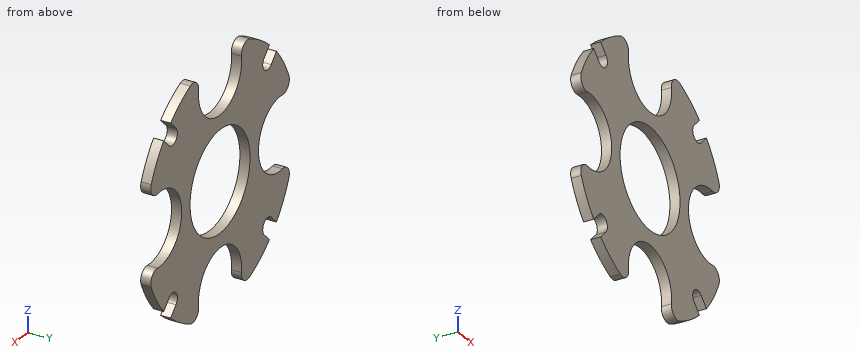
```python
from build123d import *

# Parameters (mm, degrees)
SKETCH4_R           = 5
BOSS_EXTRUDE1_DEPTH = 1


with BuildPart() as part:
    # Sketch4 → Boss-Extrude1 (new body)
    with BuildSketch(Plane(origin=(0, 0, 0), x_dir=(1, 0, 0), z_dir=(0, 1, 0))):
        with BuildLine():
            Line((-7.353910524, -8.520636713), (-8.236199678, -9.402925867))
            ThreePointArc((-8.236199678, -9.402925867), (-6.68048223, -10.565091442), (-4.963540243, -11.472282609))
            ThreePointArc((-4.963540243, -11.472282609), (-3.967940107, -11.355610167), (-3.573748975, -10.433956522))
            ThreePointArc((-3.573748975, -10.433956522), (0, -6.4), (3.573748975, -10.433956522))
            ThreePointArc((3.573748975, -10.433956522), (3.967940107, -11.355610167), (4.963540243, -11.472282609))
            ThreePointArc((4.963540243, -11.472282609), (6.68048223, -10.565091442), (8.236199678, -9.402925867))
            Line((8.236199678, -9.402925867), (7.353910524, -8.520636713))
            ThreePointArc((7.353910524, -8.520636713), (7.353910524, -7.353910524), (8.520636713, -7.353910524))
            Line((8.520636713, -7.353910524), (9.402925867, -8.236199678))
            ThreePointArc((9.402925867, -8.236199678), (10.565091442, -6.68048223), (11.472282609, -4.963540243))
            ThreePointArc((11.472282609, -4.963540243), (11.355610167, -3.967940107), (10.433956522, -3.573748975))
            ThreePointArc((10.433956522, -3.573748975), (6.4, 0), (10.433956522, 3.573748975))
            ThreePointArc((10.433956522, 3.573748975), (11.355610167, 3.967940107), (11.472282609, 4.963540243))
            ThreePointArc((11.472282609, 4.963540243), (10.565091442, 6.68048223), (9.402925867, 8.236199678))
            Line((9.402925867, 8.236199678), (8.520636713, 7.353910524))
            ThreePointArc((8.520636713, 7.353910524), (7.353910524, 7.353910524), (7.353910524, 8.520636713))
            Line((7.353910524, 8.520636713), (8.236199678, 9.402925867))
            ThreePointArc((8.236199678, 9.402925867), (6.68048223, 10.565091442), (4.963540243, 11.472282609))
            ThreePointArc((4.963540243, 11.472282609), (3.967940107, 11.355610167), (3.573748975, 10.433956522))
            ThreePointArc((3.573748975, 10.433956522), (0, 6.4), (-3.573748975, 10.433956522))
            ThreePointArc((-3.573748975, 10.433956522), (-3.967940107, 11.355610167), (-4.963540243, 11.472282609))
            ThreePointArc((-4.963540243, 11.472282609), (-6.68048223, 10.565091442), (-8.236199678, 9.402925867))
            Line((-8.236199678, 9.402925867), (-7.353910524, 8.520636713))
            ThreePointArc((-7.353910524, 8.520636713), (-7.353910524, 7.353910524), (-8.520636713, 7.353910524))
            Line((-8.520636713, 7.353910524), (-9.402925867, 8.236199678))
            ThreePointArc((-9.402925867, 8.236199678), (-10.565091442, 6.68048223), (-11.472282609, 4.963540243))
            ThreePointArc((-11.472282609, 4.963540243), (-11.355610167, 3.967940107), (-10.433956522, 3.573748975))
            ThreePointArc((-10.433956522, 3.573748975), (-6.4, 0), (-10.433956522, -3.573748975))
            ThreePointArc((-10.433956522, -3.573748975), (-11.355610167, -3.967940107), (-11.472282609, -4.963540243))
            ThreePointArc((-11.472282609, -4.963540243), (-10.565091442, -6.68048223), (-9.402925867, -8.236199678))
            Line((-9.402925867, -8.236199678), (-8.520636713, -7.353910524))
            ThreePointArc((-8.520636713, -7.353910524), (-7.353910524, -7.353910524), (-7.353910524, -8.520636713))
        make_face()
        with Locations(Location((0, 0, 0), (0, 0, 90))):
            Circle(SKETCH4_R, mode=Mode.SUBTRACT)
    extrude(amount=BOSS_EXTRUDE1_DEPTH)


solid = part.part
```
Source: CAD feature listing. Evaluate the final solid. Frame: model axes, mm. Coordinates: 2 decimals unless noted, no trailing zeros. Loops run counter-clockwise (first coordinate to the right, second up) from the corner with the lowest first, then second, coordinate; pieces in that order, holes last. Notation, with made-up numbers: (16.5, 79) - (45.5, 79) arc R32 ccw to (45.5, 117) - close; hole circle Ø7 at (68, 48). An arc over 180 degrees is marked (long way). Answer as CSV lines item,"result".
1. Ray query, line 1 (X direction, y = 0.35, z = 0); line 2 (Z direction, x = -7.5, y = 0.1); line 3 (Z direction, x = 7.75, y = 0.45). Return the intervals inside material, ascending.
Established:
line 1,"x = -6.4 to -5, 5 to 6.4"
line 2,"z = -10 to -8.67, -7.24 to -2.59, 2.59 to 7.24, 8.67 to 10"
line 3,"z = -9.81 to -8.92, -7.13 to -2.81, 2.81 to 7.13, 8.92 to 9.81"
2. Contact query for a flat-ended pin moving along its axis: pin 1 (1.5 mm diameter, centred on x = -7.5, z = 7.5, fed in from -Y). Output: stop coordinate, or through.
Established:
pin 1,"stops at y = 0"
3. Section B-B (x = 10). Return loops of the section in (y, z), then the cut area to 3 significant figures.
Established:
outline,"(0, -7.5) - (1, -7.5) - (1, -3.6) - (0, -3.6) - close; (0, 3.6) - (1, 3.6) - (1, 7.5) - (0, 7.5) - close"
area,"7.80 mm2"
4. Section D-D (z = -7.75). Return loops of the section in (x, y), then the cut area to 3 significant figures.
Established:
outline,"(-9.81, 0) - (-8.92, 0) - (-8.92, 1) - (-9.81, 1) - close; (-7.13, 0) - (-2.81, 0) - (-2.81, 1) - (-7.13, 1) - close; (2.81, 0) - (7.13, 0) - (7.13, 1) - (2.81, 1) - close; (8.92, 0) - (9.81, 0) - (9.81, 1) - (8.92, 1) - close"
area,"10.4 mm2"
5. Section A-A (z = 10). Return loops of the section in (x, y).
Established:
outline,"(-7.5, 0) - (-3.6, 0) - (-3.6, 1) - (-7.5, 1) - close; (3.6, 0) - (7.5, 0) - (7.5, 1) - (3.6, 1) - close"
